Read the model definition and answer for the solid it produces. Units are mm, in the model's axes. Coordinates: 2 decimals unless noted, no trailing zeros. Write each loop counter-clockwise with the first axis right and the second up, starting at its lowest first coordinate (ties: lowest second). Pieces come first, ordered by that corner, then holes. Notation, with made-up numbers: (47, 36) -> (105, 36) arc R16 cw to (105, 50) -> close; hole circle Ø7 at (-30.75, -38). An arc over 180 degrees is marked (long way). Return JSON: item names as keys, results as strings.
from build123d import *

# Parameters (mm, degrees)
SKETCH_1_W      = 300
SKETCH_1_H      = 400
EXTRUDE_1_DEPTH = 100
EXTRUDE_2_DEPTH = 6


with BuildPart() as part:
    # 草图1 → 凸台-拉伸1 (new, symmetric)
    with BuildSketch(Plane.XY):
        Rectangle(SKETCH_1_W, SKETCH_1_H)
    extrude(amount=EXTRUDE_1_DEPTH, both=True)

    # 草图2 → 凸台-拉伸2 (add)
    with BuildSketch(Plane.XY.offset(100)):
        with BuildLine():
            Line((128.030025312, 28.454220127), (128.030025312, -11.695906433))
            ThreePointArc((128.030025312, -11.695906433), (120, -19.725931745), (111.969974688, -11.695906433))
            Line((111.969974688, -11.695906433), (111.969974688, 28.454220127))
            ThreePointArc((111.969974688, 28.454220127), (120, 36.484245439), (128.030025312, 28.454220127))
        make_face()
    extrude(amount=EXTRUDE_2_DEPTH)


solid = part.part
1. The part is cut by section A-A (x = 120). Determine the outline of the cut face in (y, z), then the cut area to 3 significant figures.
Taken from the geometry:
{"outline": "(-200, -100) -> (200, -100) -> (200, 100) -> (36.48, 100) -> (36.48, 106) -> (-19.73, 106) -> (-19.73, 100) -> (-200, 100) -> close", "area": "80,300 mm2"}
2. The part is cut by section D-D (y = 145.5). Determine the outline of the cut face in (x, z), then the cut area to 3 significant figures.
Taken from the geometry:
{"outline": "(-150, -100) -> (150, -100) -> (150, 100) -> (-150, 100) -> close", "area": "60,000 mm2"}
3. The part is cut by section B-B (y = 24). Determine the outline of the cut face in (x, z), then the cut area to 3 significant figures.
Taken from the geometry:
{"outline": "(-150, -100) -> (150, -100) -> (150, 100) -> (128.03, 100) -> (128.03, 106) -> (111.97, 106) -> (111.97, 100) -> (-150, 100) -> close", "area": "60,100 mm2"}
4. The part is cut by section C-C (x = 49). Determine the outline of the cut face in (y, z).
Taken from the geometry:
{"outline": "(-200, -100) -> (200, -100) -> (200, 100) -> (-200, 100) -> close"}
5. Consider L1, parallel to Z at x = 33, y = -51.5. Determine where the line is inside the solid, lowest interval first.
Taken from the geometry:
{"L1": "z = -100 to 100"}
6. Flat-ended cylindrical pins translate along their axes: pin 1 Ø3 at (y, z) = (2, 103) entering from -X; pin 2 Ø3 at (y, z) = (14, 104.5) entering from +X; pin 3 Ø4 at (x, y) = (-76.5, -126) entering from +Z. Find the tip coordinate at first contact, or state that the pin passes through.
Taken from the geometry:
{"pin 1": "stops at x = 111.97", "pin 2": "stops at x = 128.03", "pin 3": "stops at z = 100"}
